```python
from build123d import *

# Parameters (mm, degrees)
SKETCH_2_R          = 2
CUT_EXTRUDE_1_DEPTH = 1
SKETCH_3_R          = 11.13
CUT_EXTRUDE_2_DEPTH = 10


with BuildPart() as part:
    # 草图1 → 旋转3 (revolve)
    with BuildSketch(Plane.XY):
        with BuildLine():
            Line((0, 13), (0, 12))
            Line((0, 12), (16, 12))
            ThreePointArc((16, 12), (18.828427125, 10.828427125), (20, 8))
            Line((20, 8), (20, 0))
            ThreePointArc((20, 0), (20.292893219, -0.707106781), (21, -1))
            Line((21, -1), (31, -1))
            Line((31, -1), (31, 0))
            Line((31, 0), (22, 0))
            ThreePointArc((22, 0), (21.292893219, 0.292893219), (21, 1))
            Line((21, 1), (21, 9))
            ThreePointArc((21, 9), (19.828427125, 11.828427125), (17, 13))
            Line((17, 13), (0, 13))
        make_face()
    revolve(axis=Axis((0, 0, 0), (0, 1, 0)))

    # 草图2 → 切除-拉伸1 (cut)
    with BuildSketch(Plane(origin=(0, 0, 0), x_dir=(1, 0, 0), z_dir=(0, 1, 0))):
        with Locations(Location((0, 25, 0), (0, 0, 180))):
            Circle(SKETCH_2_R)
        with Locations(Location((25, 0, 0), (0, 0, 180))):
            Circle(SKETCH_2_R)
        with Locations(Location((0, -25, 0), (0, 0, 180))):
            Circle(SKETCH_2_R)
        with Locations(Location((-25, 0, 0), (0, 0, 180))):
            Circle(SKETCH_2_R)
    extrude(amount=-CUT_EXTRUDE_1_DEPTH, mode=Mode.SUBTRACT)

    # 草图3 → 切除-拉伸2 (cut)
    with BuildSketch(Plane(origin=(0, 13, 0), x_dir=(1, 0, 0), z_dir=(0, 1, 0))):
        with Locations(Location((0, 0, 0), (0, 0, 180))):
            Circle(SKETCH_3_R)
    extrude(amount=-CUT_EXTRUDE_2_DEPTH, mode=Mode.SUBTRACT)


solid = part.part
```
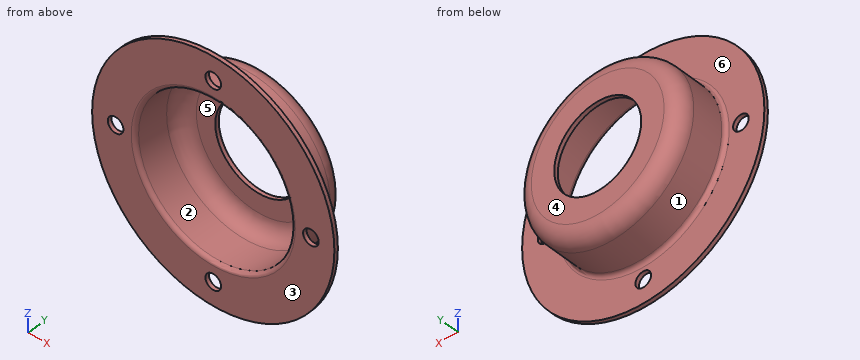
The listing builds one solid part. Answer for the finished solid, in the listing's coordinates (mm). Face numbers are marked on the shaded views. A direction names the side the tool comes from. Give positions to 0.01 mm unless a question says otherwise; leave off trailing zeros. Order: outer loops, then holes, each group sorted by start corner. A loop starts at its lowest first (then second) coordinate and runs counter-clockwise, first axis right, second up. Notation, with made-up numbers: (13.25, 36.25) - (37.25, 36.25) arc R22 cw to (37.25, 42.25) - close; hole circle Ø6 at (65.5, -14). An arc over 180 degrees is marked (long way). Use one line per item in the form item = value. Start each with the question number.
(1) Consider line 1 (Z direction, x = 0, y = -0.35); line 2 (X direction, y = 9.5, z = -14); line 3 (X direction, y = 8.25, z = 8.5). Determine where each line is inside the solid, lowest interval first. Write a range as from..to.
(2) The mould has two halves that part along Z. Classify the marked faces 1, 2 and 3: released by +Z, released by -Z, zero draft, split by the parting line, or undercut.
(3) A cutting plane is placed at A-A, the plane z = 0. State how many separate pieces and enclosed holes the cut face has, then the cut area to 3 significant figures.
(4) A cutting plane is placed at C-C, the plane x = -24. Write down the section's boundary in (y, z).
(5) Flat-ended cylindrical pins translate along their axes: pin 1 Ø1.5 at (x, y) = (12, 4) entering from +Z; pin 2 Ø6.5 at (x, z) = (25, 0) entering from +Y; pin 3 Ø1 at (x, z) = (10, 1) entering from -Y; pin 4 Ø1 at (y, z) = (3, -8.5) entering from -X. Find the tip coordinate at first contact, or state that the pin passes through.
(6) For the marked faces 4, 5 and 6, determine the directions among +Z, -Z, +X, -X, +Y, -Y from which every point of the face is accessible in a straight line to the end or side of a thin tool.
(7) A cutting plane is placed at D-D, the plane z = -25. Write down the section's boundary in (x, y).
Ans:
q1.line_1 = -31..-27, -23..-20.06, 20.06..23, 27..31
q1.line_2 = -15.61..-13.87, 13.87..15.61
q1.line_3 = -19.2..-18.1, 18.1..19.2
q2.face_1 = split by the parting line
q2.face_2 = undercut
q2.face_3 = zero draft
q3.separate_pieces = 4
q3.enclosed_holes = 0
q3.area = 57.7 mm^2
q4.outline = (-1, -19.62) - (0, -19.62) - (0, -1.73) - (-1, -1.73) - close; (-1, 1.73) - (0, 1.73) - (0, 19.62) - (-1, 19.62) - close
q5.pin_1 = 17.73
q5.pin_2 = 0.03
q5.pin_3 = through
q5.pin_4 = -19.42
q6.face_4 = +Z, -Z, +X, -X, +Y
q6.face_5 = -Y
q6.face_6 = +Y
q7.outline = (-18.33, -1) - (-2, -1) - (-2, 0) - (-18.33, 0) - close; (2, -1) - (18.33, -1) - (18.33, 0) - (2, 0) - close
